Part model, mm, in its own coordinate system. A direction names the side the tool comes from. Round coordinates to 2 decimals unless told otherwise and drop trailing zeros. Write each loop counter-clockwise with the first axis right and the second up, starting at its lowest first coordinate (ties: lowest second). Pieces come first, ordered by that corner, then holes.
from build123d import *

# Parameters (mm, degrees)
CHAMFER1_SIZE = 0.5


with BuildPart() as part:
    # Sketch1 → Revolve8 (revolve)
    with BuildSketch(Plane.XY, mode=Mode.PRIVATE) as revolve8_sk:
        Polygon((20.861200947, -54.530577635), (24.233987709, -54.530577635), (24.233987709, -72.330577635), (11.733987709, -72.330577635), (11.733987709, -70.330577635), (14.233987709, -70.330577635), (14.233987709, -62.330577635), (19.233987709, -62.330577635), (19.233987709, -60.530577635), (20.861200947, -60.530577635), align=None)
    revolve(revolve8_sk.sketch.rotate(Axis((24.233987709, -52.030577635, 0), (0, -1, 0)), 270), axis=Axis((24.233987709, -52.030577635, 0), (0, -1, 0)))

    # Chamfer1
    chamfer1_edges = [part.edges().sort_by_distance(p)[0] for p in [
        (24.233987709, -54.530577635, -3.372786762),
        (24.233987709, -60.530577635, -5),
    ]]
    chamfer(chamfer1_edges, length=CHAMFER1_SIZE)


solid = part.part
Q1. Drop flat-ended pins along their axis: P1, Ø8, axis at x = 31, y = -56.5, coming from the -Z side; P2, Ø1, axis at y = -64.5, z = 6.5, coming from the -X side; P3, Ø3, axis at y = -65.5, z = -4, coming from the -X side. Give the stop position or say it passes through.
Q2. Saw through at C-C, the plane z = -7. Write the cut outline in (x, y), and give its area (3 significant figures).
Q3. Tool access for faces 1 (the flat face through (21, -60.531, 2)), 2 (the flat face through (24, -54.531, 0)): list every direction of +Z, -Z, +X, -X, +Y, -Y with a clear straight run to the whole face (end or side of a thin tool).
Q4. Saw through at B-B, the plane x = 17.5. Write the cut outline in (y, z).
Q5. Saw through at D-D, the plane y = -59.25. Write the cut outline in (x, z), and give its area (3 significant figures).
Q6. Saw through at A-A, the plane z = 0. Write the cut outline in (x, y).
Q7. Wall check: line 1 (Y direction, x = 29, z = -4.75); line 2 (Y direction, x = 13, z = -4.75); line 3 (X direction, y = -57.5, z = 0). Give the ranges that are in metal, low to high.
Computed:
1. P1: stops at z = -1.93
1. P2: stops at x = 16.23
1. P3: stops at x = 14.55
2. outline: (13.88, -72.33) - (34.59, -72.33) - (34.59, -70.33) - (31.38, -70.33) - (31.38, -62.33) - (17.09, -62.33) - (17.09, -70.33) - (13.88, -70.33) - close
2. area: 156 mm2
3. face 1: +Y
3. face 2: +Z, -Z, +X, -X, +Y
4. outline: (-72.33, -10.53) - (-70.33, -10.53) - (-70.33, -7.39) - (-62.33, -7.39) - (-62.33, 7.39) - (-70.33, 7.39) - (-70.33, 10.53) - (-72.33, 10.53) - close
5. outline: circle Ø6.75 at (24.23, 0)
5. area: 35.7 mm2
6. outline: (11.73, -72.33) - (36.73, -72.33) - (36.73, -70.33) - (34.23, -70.33) - (34.23, -62.33) - (29.23, -62.33) - (29.23, -61.03) - (28.73, -60.53) - (27.61, -60.53) - (27.61, -55.03) - (27.11, -54.53) - (21.36, -54.53) - (20.86, -55.03) - (20.86, -60.53) - (19.73, -60.53) - (19.23, -61.03) - (19.23, -62.33) - (14.23, -62.33) - (14.23, -70.33) - (11.73, -70.33) - close
7. line 1: y = -72.33 to -62.33
7. line 2: y = -72.33 to -70.33
7. line 3: x = 20.86 to 27.61
